from build123d import *

# Parameters (mm, degrees)
BOSS_EXTRUDE1_DEPTH = 16
SKETCH2_R           = 5
CUT_EXTRUDE1_DEPTH  = 16
SKETCH3_R           = 8
BOSS_EXTRUDE2_DEPTH = 32
BOSS_EXTRUDE3_START = -32
SKETCH4_R           = 8
BOSS_EXTRUDE3_DEPTH = 32
SKETCH5_W           = 30
SKETCH5_H           = 8
CUT_EXTRUDE2_DEPTH  = 38
SKETCH6_R           = 4
CUT_EXTRUDE3_DEPTH  = 38


with BuildPart() as part:
    # Sketch1 → Boss-Extrude1 (new body)
    with BuildSketch(Plane.XY):
        with BuildLine():
            Line((0, 8), (-97.477609689, 8))
            Line((-97.477609689, 8), (-160.943552052, 52.439331262))
            ThreePointArc((-160.943552052, 52.439331262), (-172.085379897, 50.474726399), (-170.120775034, 39.332898554))
            Line((-170.120775034, 39.332898554), (-102.522390311, -8))
            Line((-102.522390311, -8), (0, -8))
            ThreePointArc((0, -8), (8, 0), (0, 8))
        make_face()
    extrude(amount=BOSS_EXTRUDE1_DEPTH)

    # Sketch2 → Cut-Extrude1 (cut)
    with BuildSketch(Plane.XY.offset(16)):
        Circle(SKETCH2_R)
    extrude(amount=-CUT_EXTRUDE1_DEPTH, mode=Mode.SUBTRACT)

    # Sketch3 → Boss-Extrude2 (add)
    with BuildSketch(Plane(origin=(0, 0, 0), x_dir=(-1, 0, 0), z_dir=(0, 0, -1))):
        with Locations((100, 0)):
            Circle(SKETCH3_R)
    extrude(amount=-BOSS_EXTRUDE2_DEPTH)

    # Sketch4 → Boss-Extrude3 (add)
    with BuildSketch(Plane.XY.offset(16).offset(BOSS_EXTRUDE3_START)):
        with Locations(Location((-165.532163543, 45.886114908, 0), (0, 0, 235))):
            Circle(SKETCH4_R)
    extrude(amount=BOSS_EXTRUDE3_DEPTH)

    # Sketch5 → Cut-Extrude2 (cut)
    with BuildSketch(Plane(origin=(-37.487604325, -53.537847394, 0), x_dir=(0.819152044288991, -0.5735764363510472, 0), z_dir=(-0.5735764363510472, -0.819152044288991, 0))):
        with Locations((-161.915204429, 8)):
            Rectangle(SKETCH5_W, SKETCH5_H)
    extrude(amount=-CUT_EXTRUDE2_DEPTH, mode=Mode.SUBTRACT)

    # Sketch6 → Cut-Extrude3 (cut)
    with BuildSketch(Plane.XY.offset(16)):
        with Locations((-165.532163543, 45.886114908)):
            Circle(SKETCH6_R)
    extrude(amount=-CUT_EXTRUDE3_DEPTH, mode=Mode.SUBTRACT)


solid = part.part
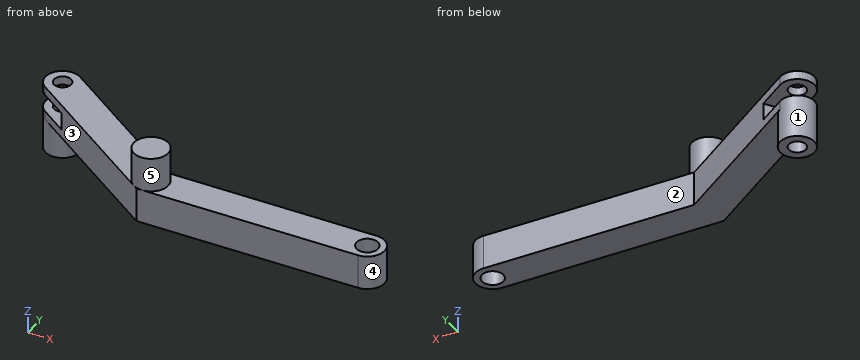
The listing builds one solid part. Answer for the finished solid, in the listing's coordinates (mm). Face numbers are marked on the shaded views. A direction names the side the tool comes from. Coordinates: 2 decimals unless noted, no trailing zeros. Order: outer loops, then holes, each group sorted by start corner. A loop starts at its lowest first (then second) coordinate and runs counter-clockwise, first axis right, second up.
Q1. A cutting plane is placed at C-C, the plane z = -3.5. Write down the section's boundary in (x, y).
Q2. A cutting plane is placed at B-B, the plane x = -17. Write down the section's boundary in (y, z).
Q3. A cutting plane is placed at A-A, the plane y = -3. Write down the section's boundary in (x, z).
Q4. Consider line 1 (Z direction, x = -120, y = 6); line 2 (Y direction, x = -17, z = 2.5); line 3 (X direction, y = -1, z = 0.5). Determine where each line is inside the solid, lowest interval first.
Q5. Given P1, Ø13, axis at x = -42.5, z = 7, coming from the +Y side; P2, Ø7, axis at x = -158, y = 44, coming from the +Z side; P3, Ø13, axis at x = 0, y = 0, coming from the -Z side, each flat-ended and moving along its own axis, determine where each tip first touches the part or whether it passes through.
Q6. A cutting plane is placed at D-D, the plane y = 33.5. Write down the section's boundary in (x, z).
Q7. Which of the six approach directions +Z, -Z, +X, -X, +Y, -Y give full straight-line access (tool end or side, diameter ignored) to the marked faces 1, 2, 3, 4 and 5?
Answers follow:
1. outline: circle Ø16 at (-165.53, 45.89); hole circle Ø8 at (-165.53, 45.89)
2. outline: (-8, 0) - (8, 0) - (8, 16) - (-8, 16) - close
3. outline: (-109.66, 0) - (-4, 0) - (-4, 16) - (-92.58, 16) - (-92.58, 32) - (-107.42, 32) - (-107.42, 16) - (-109.66, 16) - close; (4, 0) - (7.42, 0) - (7.42, 16) - (4, 16) - close
4. line 1: z = 0 to 16
4. line 2: y = -8 to 8
4. line 3: x = -112.52 to -4.9, 4.9 to 7.94
5. P1: stops at y = 8
5. P2: stops at z = 16
5. P3: stops at z = 0
6. outline: (-161.79, 0) - (-133.9, 0) - (-133.9, 16) - (-161.79, 16) - (-161.79, 12) - (-155.89, 12) - (-155.89, 4) - (-161.79, 4) - close
7. face 1: -Z
7. face 2: +Z, -Z, +X, +Y
7. face 3: +Z, -Z, -X, -Y
7. face 4: +Z, -Z, +X
7. face 5: +Z
